CAD build for the part. Positions are in the model's coordinates, mm. Face numbers are marked on the shaded views. A direction names the side the tool comes from. Round coordinates to 2 decimals unless told otherwise and drop trailing zeros. Loops run counter-clockwise (first coordinate to the right, second up) from the corner with the lowest first, then second, coordinate; pieces in that order, holes last.
```python
from build123d import *

# Parameters (mm, degrees)
SKETCH1_W             = 195
SKETCH1_H             = 14
EXTRUDE_THIN1_DEPTH   = 10
M4_TAPPED_HOLE1_D     = 3.3
M4_TAPPED_HOLE1_DEPTH = 10.1
M4_TAPPED_HOLE1_TIP   = 0.991420021
M4_TAPPED_HOLE2_D     = 3.3
M4_TAPPED_HOLE2_DEPTH = 10.1
M4_TAPPED_HOLE2_TIP   = 0.991420021
M5_TAPPED_HOLE1_D     = 4.2
SKETCH9_R             = 4.4
CUT_EXTRUDE1_DEPTH    = 3
SKETCH10_W            = 160
SKETCH10_H            = 3.5
CUT_EXTRUDE2_DEPTH    = 196.757503049


with BuildPart() as part:
    # Sketch1 → Extrude-Thin1 (new, symmetric)
    with BuildSketch(Plane.XY):
        with Locations((-97.5, 7)):
            Rectangle(SKETCH1_W, SKETCH1_H)
    extrude(amount=EXTRUDE_THIN1_DEPTH, both=True)

    # M4 Tapped Hole1
    with Locations(Plane.ZY.offset(195)):
        with Locations((-6, 7), (6, 7)):
            Hole(M4_TAPPED_HOLE1_D / 2, depth=M4_TAPPED_HOLE1_DEPTH)
            with Locations((0, 0, -(M4_TAPPED_HOLE1_DEPTH + M4_TAPPED_HOLE1_TIP / 2))):  # 118° drill point
                Cone(0, M4_TAPPED_HOLE1_D / 2, M4_TAPPED_HOLE1_TIP, mode=Mode.SUBTRACT)

    # M4 Tapped Hole2
    with Locations(Plane(origin=(0, 0, 0), x_dir=(0, 0, -1), z_dir=(1, 0, 0))):
        with Locations((-6, 7), (6, 7)):
            Hole(M4_TAPPED_HOLE2_D / 2, depth=M4_TAPPED_HOLE2_DEPTH)
            with Locations((0, 0, -(M4_TAPPED_HOLE2_DEPTH + M4_TAPPED_HOLE2_TIP / 2))):  # 118° drill point
                Cone(0, M4_TAPPED_HOLE2_D / 2, M4_TAPPED_HOLE2_TIP, mode=Mode.SUBTRACT)

    # M5 Tapped Hole1 (through all)
    with Locations(Plane(origin=(0, 14, 0), x_dir=(1, 0, 0), z_dir=(0, 1, 0))):
        with Locations((-146, -3.5), (-85, -3.5), (-24, -3.5)):
            Hole(M5_TAPPED_HOLE1_D / 2)

    # Sketch9 → Cut-Extrude1 (cut)
    with BuildSketch(Plane(origin=(0, 14, 0), x_dir=(1, 0, 0), z_dir=(0, 1, 0))):
        with Locations(Location((-146, -3.5, 0), (0, 0, 180))):
            Circle(SKETCH9_R)
        with Locations(Location((-85, -3.5, 0), (0, 0, 180))):
            Circle(SKETCH9_R)
        with Locations(Location((-24, -3.5, 0), (0, 0, 180))):
            Circle(SKETCH9_R)
    extrude(amount=-CUT_EXTRUDE1_DEPTH, mode=Mode.SUBTRACT)

    # Sketch10 → Cut-Extrude2 (cut, through all)
    with BuildSketch(Plane(origin=(0, 14, 0), x_dir=(1, 0, 0), z_dir=(0, 1, 0))):
        with Locations((-97.5, 8.25)):
            Rectangle(SKETCH10_W, SKETCH10_H)
    extrude(amount=-CUT_EXTRUDE2_DEPTH, mode=Mode.SUBTRACT)


solid = part.part
```
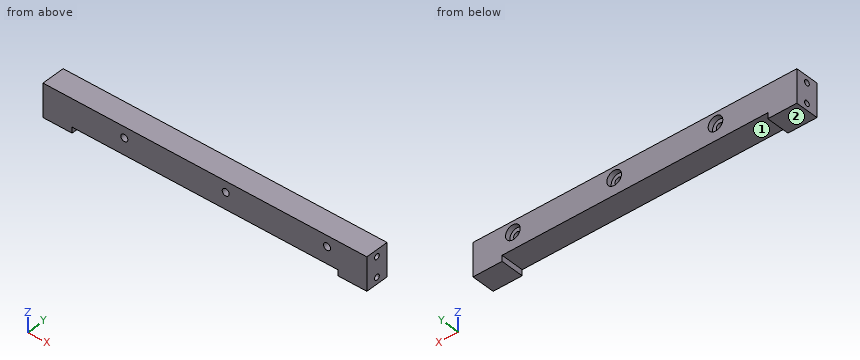
Item 1: Cut at B-B, the plane x = -85.5. Give the cut face in (y, z).
Answers follow:
outline: (0, -6.5) - (14, -6.5) - (14, -0.87) - (11, -0.87) - (11, 1.46) - (0, 1.46) - close; (0, 5.54) - (11, 5.54) - (11, 7.87) - (14, 7.87) - (14, 10) - (0, 10) - close
Item 2: Flat gauge pins, fed straight in: P1, Ø5.5, axis at x = -85, z = 3.5, coming from the -Y side; P2, Ø4, axis at x = -146, z = 3.5, coming from the -Y side; P3, Ø3, axis at y = 7, z = 6, coming from the +X side; P4, Ø1, axis at x = -46, y = 12, coming from the -Z side. Where does each tip first touch, or does it go through?
Answers follow:
P1: stops at y = 0
P2: passes through
P3: stops at x = -10.19
P4: stops at z = -6.5
Item 3: 3-axis set-ups, long thin cutter, end or side, ignore diameter. For the marked faces 1 and 2: which of +Z, -Z, +X, -X, +Y, -Y reach the whole face in a straight line?
Answers follow:
face 1: -Z, +Y, -Y
face 2: -Z, +X, -X, +Y, -Y
Item 4: Cut at A-A, the plane x = -146. Give the cut face in (y, z).
Answers follow:
outline: (0, -6.5) - (14, -6.5) - (14, -0.9) - (11, -0.9) - (11, 1.4) - (0, 1.4) - close; (0, 5.6) - (11, 5.6) - (11, 7.9) - (14, 7.9) - (14, 10) - (0, 10) - close
Item 5: Probe line 1 (Z direction, x = -2.5, y = 7); line 2 (Y direction, x = -4.5, z = -6); line 3 (Z direction, x = -24, y = 5). List the from-to ranges inside material, lowest first.
Answers follow:
line 1: z = -10 to -7.65, -4.35 to 4.35, 7.65 to 10
line 2: y = 0 to 5.35, 8.65 to 14
line 3: z = -6.5 to 1.4, 5.6 to 10
